```python
from build123d import *

# Parameters (mm, degrees)
SKETCH_2_W             = 185
SKETCH_2_H             = 90
EXTRUDE_1_DEPTH        = 8
SKETCH_4_W             = 115
SKETCH_4_H             = 15
CUT_EXTRUDE_7_DEPTH    = 104.175820811
SKETCH_5_R             = 26
CUT_EXTRUDE_8_DEPTH    = 104.175820811
HOLE_WIZARD_M5_1_D     = 4.2
SKETCH_10_R            = 20
CUT_EXTRUDE_9_DEPTH    = 104.175820811
CUT_EXTRUDE_15_DEPTH   = 6
CUT_EXTRUDE_16_DEPTH   = 104.040040761
HOLE_WIZARD_M4_1_D     = 3.3
HOLE_WIZARD_M4_1_DEPTH = 12
HOLE_WIZARD_M4_1_TIP   = 0.991420021
HOLE_WIZARD_M4_2_D     = 3.3
HOLE_WIZARD_M4_2_DEPTH = 12
HOLE_WIZARD_M4_2_TIP   = 0.991420021
CHAMFER_1_SIZE         = 25
CHAMFER_2_SIZE         = 2
FILLET_1_R             = 10


with BuildPart() as part:
    # 草图2 → 凸台-拉伸1 (new body)
    with BuildSketch(Plane(origin=(0, 0, 0), x_dir=(1, 0, 0), z_dir=(0, 1, 0))):
        Rectangle(SKETCH_2_W, SKETCH_2_H)
    extrude(amount=EXTRUDE_1_DEPTH)

    # 草图4 → 切除-拉伸7 (cut, through all)
    with BuildSketch(Plane(origin=(0, 8, 0), x_dir=(1, 0, 0), z_dir=(0, 1, 0))):
        with Locations((35, -37.5)):
            Rectangle(SKETCH_4_W, SKETCH_4_H)
    extrude(amount=-CUT_EXTRUDE_7_DEPTH, mode=Mode.SUBTRACT)

    # 草图5 → 切除-拉伸8 (cut, through all)
    with BuildSketch(Plane(origin=(0, 8, 0), x_dir=(1, 0, 0), z_dir=(0, 1, 0))):
        with Locations(Location((-57.5, -10, 0), (0, 0, 270))):
            Circle(SKETCH_5_R)
    extrude(amount=-CUT_EXTRUDE_8_DEPTH, mode=Mode.SUBTRACT)

    # M5 螺纹孔1 (through all)
    with Locations(Plane(origin=(0, 8, 0), x_dir=(1, 0, 0), z_dir=(0, 1, 0))):
        with Locations((-82.248737342, 14.748737342), (-32.751262658, 14.748737342), (-32.751262658, -34.748737342), (-82.248737342, -34.748737342), (-57.5, -10)):
            Hole(HOLE_WIZARD_M5_1_D / 2)

    # 草图10 → 切除-拉伸9 (cut, through all)
    with BuildSketch(Plane(origin=(0, 8, 0), x_dir=(1, 0, 0), z_dir=(0, 1, 0))):
        with Locations(Location((52.5, 7.5, 0), (0, 0, 270))):
            Circle(SKETCH_10_R)
    extrude(amount=-CUT_EXTRUDE_9_DEPTH, mode=Mode.SUBTRACT)

    # 草图15 → 切除-拉伸15 (cut)
    with BuildSketch(Plane(origin=(0, 8, 0), x_dir=(1, 0, 0), z_dir=(0, 1, 0))):
        with BuildLine():
            Line((73, -13), (83, -13))
            ThreePointArc((83, -13), (88, -18), (83, -23))
            Line((83, -23), (73, -23))
            ThreePointArc((73, -23), (68, -18), (73, -13))
        make_face()
        with BuildLine():
            Line((73, 28), (83, 28))
            ThreePointArc((83, 28), (88, 33), (83, 38))
            Line((83, 38), (73, 38))
            ThreePointArc((73, 38), (68, 33), (73, 28))
        make_face()
        with BuildLine():
            Line((22, -13), (32, -13))
            ThreePointArc((32, -13), (37, -18), (32, -23))
            Line((32, -23), (22, -23))
            ThreePointArc((22, -23), (17, -18), (22, -13))
        make_face()
        with BuildLine():
            Line((22, 28), (32, 28))
            ThreePointArc((32, 28), (37, 33), (32, 38))
            Line((32, 38), (22, 38))
            ThreePointArc((22, 38), (17, 33), (22, 28))
        make_face()
    extrude(amount=-CUT_EXTRUDE_15_DEPTH, mode=Mode.SUBTRACT)

    # 草图16 → 切除-拉伸16 (cut, through all)
    with BuildSketch(Plane(origin=(0, 2, 0), x_dir=(1, 0, 0), z_dir=(0, 1, 0))):
        with BuildLine():
            Line((73, -15), (83, -15))
            ThreePointArc((83, -15), (86, -18), (83, -21))
            Line((83, -21), (73, -21))
            ThreePointArc((73, -21), (70, -18), (73, -15))
        make_face()
        with BuildLine():
            Line((73, 30), (83, 30))
            ThreePointArc((83, 30), (86, 33), (83, 36))
            Line((83, 36), (73, 36))
            ThreePointArc((73, 36), (70, 33), (73, 30))
        make_face()
        with BuildLine():
            Line((22, -15), (32, -15))
            ThreePointArc((32, -15), (35, -18), (32, -21))
            Line((32, -21), (22, -21))
            ThreePointArc((22, -21), (19, -18), (22, -15))
        make_face()
        with BuildLine():
            Line((22, 30), (32, 30))
            ThreePointArc((32, 30), (35, 33), (32, 36))
            Line((32, 36), (22, 36))
            ThreePointArc((22, 36), (19, 33), (22, 30))
        make_face()
    extrude(amount=-CUT_EXTRUDE_16_DEPTH, mode=Mode.SUBTRACT)

    # M4 螺纹孔1
    with Locations(Plane(origin=(0, 0, -45), x_dir=(-1, 0, 0), z_dir=(0, 0, -1))):
        with Locations((-52.5, 4), (52.5, 4)):
            Hole(HOLE_WIZARD_M4_1_D / 2, depth=HOLE_WIZARD_M4_1_DEPTH)
            with Locations((0, 0, -(HOLE_WIZARD_M4_1_DEPTH + HOLE_WIZARD_M4_1_TIP / 2))):  # 118° drill point
                Cone(0, HOLE_WIZARD_M4_1_D / 2, HOLE_WIZARD_M4_1_TIP, mode=Mode.SUBTRACT)

    # M4 螺纹孔2
    with Locations(Plane.XY.offset(45)):
        with Locations((-52.5, 4)):
            Hole(HOLE_WIZARD_M4_2_D / 2, depth=HOLE_WIZARD_M4_2_DEPTH)
            with Locations((0, 0, -(HOLE_WIZARD_M4_2_DEPTH + HOLE_WIZARD_M4_2_TIP / 2))):  # 118° drill point
                Cone(0, HOLE_WIZARD_M4_2_D / 2, HOLE_WIZARD_M4_2_TIP, mode=Mode.SUBTRACT)

    # 倒角1
    chamfer_1_edges = [part.edges().sort_by_distance(p)[0] for p in [
        (-92.5, 4, -45),
    ]]
    chamfer(chamfer_1_edges, length=CHAMFER_1_SIZE)

    # 倒角2
    chamfer_2_edges = [part.edges().sort_by_distance(p)[0] for p in [
        (92.5, 4, 30),
        (-22.5, 4, 45),
        (92.5, 4, -45),
    ]]
    chamfer(chamfer_2_edges, length=CHAMFER_2_SIZE)

    # 圆角1
    fillet_1_edges = [part.edges().sort_by_distance(p)[0] for p in [
        (-22.5, 4, 30),
    ]]
    fillet(fillet_1_edges, radius=FILLET_1_R)


solid = part.part
```
Work out the finished part from the listing and answer in its coordinate system (mm). A direction names the side the tool comes from. Give positions to 0.01 mm unless a question says otherwise; leave off trailing zeros. Loops run counter-clockwise (first coordinate to the right, second up) from the corner with the lowest first, then second, coordinate; pieces in that order, holes last. Notation, with made-up numbers: (83, 40) -> (94, 40) arc R17 ccw to (94, 50) -> close; hole circle Ø2 at (4.25, 41.25). An arc over 180 degrees is marked (long way). Write item = value, one per line. Start each with the question number.
(1) Find the intervals of material crossed by probe 1 along Z at (x, y) = (22.5, 7.25); probe 2 along X at (y, z) = (7, 10.5); probe 3 along X at (y, z) = (3.5, 8), in increasing order. Write a range as from..to.
(2) The mould has two halves that part along X. Classify faces 4 (the cylindrical face through (37, 5, 18)), 5 (the cylindrical face through (-19.65, 3.94, 33.01)), 6 (the flat face through (38, 4, 30)): +X half, -X half, draft (parallel to the pull), parting line (faces both ways), or undercut.
(3) Find section C-C on z = -4. Give the vertices of the cut face in (x, y), and give its area (3 significant figures).
(4) Find section D-D on z = -23. Give the vertices of the cut face in (x, y).
(5) Which of the six approach directions +Z, -Z, +X, -X, +Y, -Y give full straight-line access (tool end or side, diameter ignored) to faces 1 (the cylindrical face through (50.85, 4.07, -38.92)), 2 (the cylindrical face through (-81.975, 3.944, 32.667)), 3 (the cylindrical face through (37, 5, -33))?
(6) Given pin 1 Ø1.8 at (x, y) = (27, 3.5) entering from +Z; pin 2 Ø5 at (x, z) = (42, 6) entering from +Y; pin 3 Ø3 at (x, y) = (-52.5, 4) entering from +Z, each flat-ended and moving along its own axis, determine where each tip first touches the part or whether it passes through.
(7) Find section B-B on x = -57.5. Give the vertices of the cut face in (y, z).
(8) Find section A-A on x = 77. Give the vertices of the cut face in (y, z).
From the geometry:
q1.probe_1 = -45..-38, -28..13, 23..30
q1.probe_2 = -92.5..-83.5, -31.5..43.78, 61.22..92.5
q1.probe_3 = -92.5..-83.42, -31.58..39.86, 65.14..92.5
q2.face_4 = undercut
q2.face_5 = +X half
q2.face_6 = draft
q3.outline = (-92.5, 0) -> (-79.41, 0) -> (-79.41, 8) -> (-92.5, 8) -> close; (-35.59, 0) -> (32.81, 0) -> (32.81, 8) -> (-35.59, 8) -> close; (72.19, 0) -> (92.5, 0) -> (92.5, 8) -> (72.19, 8) -> close
q3.area = 814 mm^2
q4.outline = (-89.5, 0) -> (39.86, 0) -> (39.86, 8) -> (-89.5, 8) -> close; (65.14, 0) -> (92.5, 0) -> (92.5, 8) -> (65.14, 8) -> close
q5.face_1 = -Z
q5.face_2 = +Y, -Y
q5.face_3 = +Y
q6.pin_1 = 30
q6.pin_2 = through
q6.pin_3 = -15.17
q7.outline = (0, -45) -> (8, -45) -> (8, -16) -> (0, -16) -> close; (0, 36) -> (8, 36) -> (8, 45) -> (0, 45) -> close
q8.outline = (0, -45) -> (8, -45) -> (8, -38) -> (2, -38) -> (2, -36) -> (0, -36) -> close; (0, -30) -> (2, -30) -> (2, -28) -> (8, -28) -> (8, 13) -> (2, 13) -> (2, 15) -> (0, 15) -> close; (0, 21) -> (2, 21) -> (2, 23) -> (8, 23) -> (8, 30) -> (0, 30) -> close
